from build123d import *

# Parameters (mm, degrees)
BOSS_EXTRUDE1_DEPTH = 13
SKETCH2_R           = 3.5
SKETCH2_R_2         = 2.5
CUT_EXTRUDE1_DEPTH  = 26
SKETCH3_R           = 5.25
CUT_EXTRUDE2_DEPTH  = 6


with BuildPart() as part:
    # Sketch1 → Boss-Extrude1 (new, symmetric)
    with BuildSketch(Plane.XY):
        Polygon((55.168145317, 40.706551648), (57.168145317, 42.706551648), (57.168145317, 46.706551648), (45.168145317, 48.706551648), (35.15033873, 48.706551648), (35.15033873, 14.706551648), (35.15033873, 8.706551648), (45.168145317, 8.706551648), (45.168145317, 38.706551648), (43.168145317, 40.706551648), (45.168145317, 42.706551648), (47.168145317, 40.706551648), align=None)
    extrude(amount=BOSS_EXTRUDE1_DEPTH, both=True)

    # Sketch2 → Cut-Extrude1 (cut)
    with BuildSketch(Plane(origin=(45.168145317, 0, 0), x_dir=(0, 0, -1), z_dir=(1, 0, 0))):
        with Locations((-5, 17.706551648)):
            Circle(SKETCH2_R)
        with Locations((5, 31.706551648)):
            Circle(SKETCH2_R)
        with Locations((5, 17.706551648)):
            Circle(SKETCH2_R_2)
        with Locations((-5, 31.706551648)):
            Circle(SKETCH2_R_2)
    extrude(amount=-CUT_EXTRUDE1_DEPTH, mode=Mode.SUBTRACT)

    # Sketch3 → Cut-Extrude2 (cut)
    with BuildSketch(Plane(origin=(45.168145317, 0, 0), x_dir=(0, 0, -1), z_dir=(1, 0, 0))):
        with Locations((5, 31.706551648)):
            Circle(SKETCH3_R)
        with Locations((-5, 17.706551648)):
            Circle(SKETCH3_R)
    extrude(amount=-CUT_EXTRUDE2_DEPTH, mode=Mode.SUBTRACT)


solid = part.part
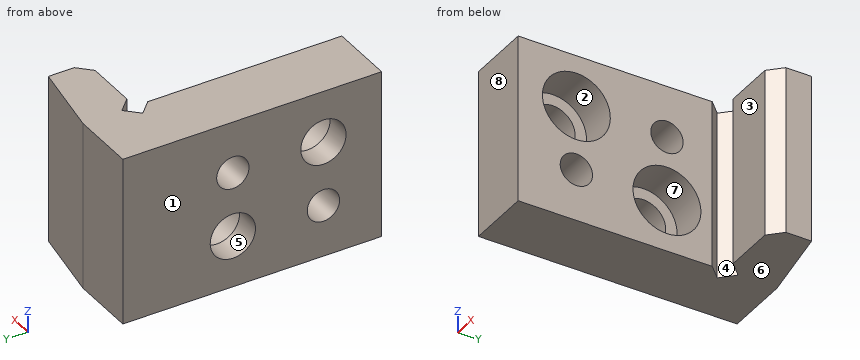
Here's how the part is built. I have some questions about the finished solid (model axes, mm). Face numbers are marked on the shaded views. A direction names the side the tool comes from. Round coordinates to 2 decimals unless told otherwise and drop trailing zeros. Write each loop counter-clockwise with the first axis right and the second up, starting at its lowest first coordinate (ties: lowest second). Pieces come first, ordered by that corner, then holes. Notation, with made-up numbers: (-20, 85.5) -> (-1, 85.5) arc R32 ccw to (-1, 113.5) -> close; hole circle Ø9 at (46, 27). An arc over 180 degrees is marked (long way). One line per item, written item: value.
1) We'd pull the mould along Z, two halves only. Please class the marked faces 6, 7 and 8: released by +Z, released by -Z, zero draft, split by the parting line, or undercut.
Filled sheet:
face 6: released by -Z
face 7: undercut
face 8: zero draft
2) For the marked faces 1, 2, 3, 4 and 5, which set-ups out of +Z, -Z, +X, -X, +Y, -Y let a thin tool reach every point of the face, with its end or its side?
Filled sheet:
face 1: +Z, -Z, -X, +Y, -Y
face 2: +X
face 3: +Z, -Z, +X, -Y
face 4: +Z, -Z
face 5: +X, -X
3) Suppose I cut it at A-A on z = 5. List the corners of the cut face in (x, y) for me.
Filled sheet:
outline: (35.15, 8.71) -> (45.17, 8.71) -> (45.17, 12.46) -> (39.17, 12.46) -> (39.17, 14.21) -> (35.15, 14.21) -> close; (35.15, 21.21) -> (39.17, 21.21) -> (39.17, 22.96) -> (45.17, 22.96) -> (45.17, 29.21) -> (35.15, 29.21) -> close; (35.15, 34.21) -> (45.17, 34.21) -> (45.17, 38.71) -> (43.17, 40.71) -> (45.17, 42.71) -> (47.17, 40.71) -> (55.17, 40.71) -> (57.17, 42.71) -> (57.17, 46.71) -> (45.17, 48.71) -> (35.15, 48.71) -> close
4) I'm going to push flat-ended pins straight in: pin 1 Ø5 at (y, z) = (28, 1) entering from +X; pin 2 Ø4 at (x, z) = (50.5, 1) entering from -Y; pin 3 Ø8.5 at (y, z) = (17.71, 5) entering from +X. Where does each tip first touch, or does it pass through?
Filled sheet:
pin 1: stops at x = 45.17
pin 2: stops at y = 40.71
pin 3: stops at x = 39.17
5) Suppose I cut it at D-D on z = -11.5. List the corners of the cut face in (x, y) for me, plus the area to 3 significant figures.
Filled sheet:
outline: (35.15, 8.71) -> (45.17, 8.71) -> (45.17, 38.71) -> (43.17, 40.71) -> (45.17, 42.71) -> (47.17, 40.71) -> (55.17, 40.71) -> (57.17, 42.71) -> (57.17, 46.71) -> (45.17, 48.71) -> (35.15, 48.71) -> close
area: 477 mm2
6) Suppose I cut it at C-C on y = 24. List the corners of the cut face in (x, z) for me, plus the area to 3 significant figures.
Filled sheet:
outline: (35.15, -13) -> (45.17, -13) -> (45.17, 13) -> (35.15, 13) -> close
area: 260 mm2
7) If I drill on line 1 (Y direction, x = 42.55, z = 5); line 2 (Y direction, x = 38, z = -5); line 3 (X direction, y = 30.5, z = -0.75), over which ranges is the centre line in solid material (lowest first)? Write a range as [from, to].
Filled sheet:
line 1: y = [8.71, 12.46], [22.96, 29.21], [34.21, 48.71]
line 2: y = [8.71, 15.21], [20.21, 28.21], [35.21, 48.71]
line 3: x = [35.15, 39.17]
8) Suppose I cut it at B-B on z = -2. List the corners of the cut face in (x, y) for me, plus the area to 3 significant figures.
Filled sheet:
outline: (35.15, 8.71) -> (45.17, 8.71) -> (45.17, 27.4) -> (39.17, 27.4) -> (39.17, 29.9) -> (35.15, 29.9) -> close; (35.15, 33.51) -> (39.17, 33.51) -> (39.17, 36.01) -> (45.17, 36.01) -> (45.17, 38.71) -> (43.17, 40.71) -> (45.17, 42.71) -> (47.17, 40.71) -> (55.17, 40.71) -> (57.17, 42.71) -> (57.17, 46.71) -> (45.17, 48.71) -> (35.15, 48.71) -> close
area: 411 mm2
